Drawing for the job (mm, zero at the part's lowest x, y, z). Coordinates: 2 decimals unless noted, no trailing zeros. Order: outer loops, then holes, each group sorted by start corner. A loop starts at its lowest first (then second) coordinate and runs counter-clockwise, first axis right, second up.
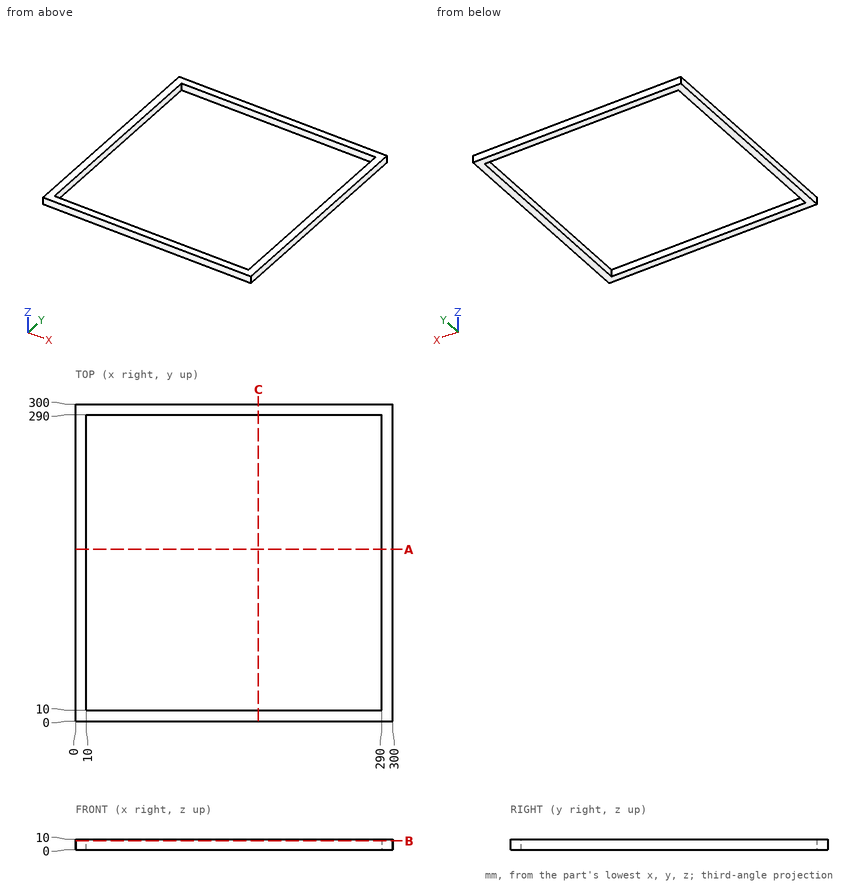
1) Slice it at A-A (y = 162.5). List the corners of the cut face in (x, z), plus the area to 3 significant figures.
2) Slice it at B-B (z = 8.25). List the corners of the cut face in (x, y), plus the area to 3 significant figures.
3) Drill centre line: probe 1 along X at (y, z) = (41.5, 2.5). Where is it in solid material? Low to high.
Worked out:
1. outline: (0, 0) - (10, 0) - (10, 10) - (0, 10) - close; (290, 0) - (300, 0) - (300, 10) - (290, 10) - close
1. area: 200 mm2
2. outline: (0, 0) - (300, 0) - (300, 300) - (0, 300) - close; hole (10, 10) - (290, 10) - (290, 290) - (10, 290) - close
2. area: 11,600 mm2
3. probe 1: x = 0 to 10, 290 to 300
